```python
from build123d import *

# Parameters (mm, degrees)
SKETCH_1_W      = 26
SKETCH_1_H      = 12
SKETCH_1_W_2    = 20
SKETCH_1_H_2    = 8
EXTRUDE_1_DEPTH = 2.5
SKETCH_2_W      = 12
SKETCH_2_H      = 9
EXTRUDE_2_DEPTH = 2.5


with BuildPart() as part:
    # 草图1 → 凸台-拉伸1 (new, symmetric)
    with BuildSketch(Plane.XY):
        Rectangle(SKETCH_1_W, SKETCH_1_H)
        Rectangle(SKETCH_1_W_2, SKETCH_1_H_2, mode=Mode.SUBTRACT)
    extrude(amount=EXTRUDE_1_DEPTH, both=True)

    # 草图2 → 凸台-拉伸2 (add, symmetric)
    with BuildSketch(Plane.XY):
        with Locations((0, -10.5)):
            Rectangle(SKETCH_2_W, SKETCH_2_H)
    extrude(amount=EXTRUDE_2_DEPTH, both=True)


solid = part.part
```
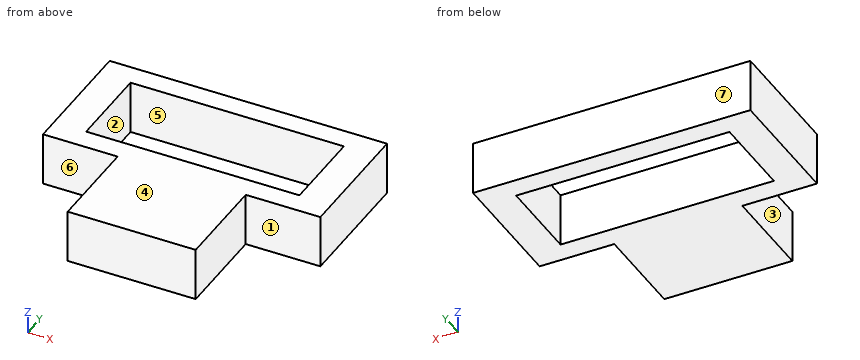
For this review, take the finished solid that the model builds, in its own axes (mm). Face numbers are marked on the shaded views. A direction names the side the tool comes from. Round coordinates to 2 decimals unless told otherwise and drop trailing zeros. Write each loop counter-clockwise with the first axis right and the second up, starting at its lowest first coordinate (ties: lowest second). Pieces come first, ordered by that corner, then holes.
1) Take a section at C-C on z = 0. Give the boundary of the cut face in (x, y), then the cut area to 3 significant figures.
Answer below:
outline: (-13, -6) - (-6, -6) - (-6, -15) - (6, -15) - (6, -6) - (13, -6) - (13, 6) - (-13, 6) - close; hole (-10, -4) - (10, -4) - (10, 4) - (-10, 4) - close
area: 260 mm2
2) Take a section at D-D on x = 10.75. Give the boundary of the cut face in (y, z).
Answer below:
outline: (-6, -2.5) - (6, -2.5) - (6, 2.5) - (-6, 2.5) - close
3) Take a section at B-B on y = 1.25. Give the boundary of the cut face in (x, z).
Answer below:
outline: (-13, -2.5) - (-10, -2.5) - (-10, 2.5) - (-13, 2.5) - close; (10, -2.5) - (13, -2.5) - (13, 2.5) - (10, 2.5) - close
4) Take a section at A-A on x = -3.75. Give the boundary of the cut face in (y, z).
Answer below:
outline: (-15, -2.5) - (-4, -2.5) - (-4, 2.5) - (-15, 2.5) - close; (4, -2.5) - (6, -2.5) - (6, 2.5) - (4, 2.5) - close
5) Machinability: for the marked faces 1, 2, 3 and 4, which of the approach directions +Z, -Z, +X, -X, +Y, -Y give a long, thin tool a straight path to every point of the face, cutting with its end or side? Answer none if there is none.
Answer below:
face 1: +Z, -Z, +X, -Y
face 2: +Z, -Z
face 3: +Z, -Z, -X, -Y
face 4: +Z, +X, -X, +Y, -Y
6) Mouldability with a two-part tool opening along Y and no side actions: class the marked faces 5, 6 and 7 as +Y half, -Y half, draft (parallel to the pull), parting line (faces both ways), or undercut.
Answer below:
face 5: undercut
face 6: -Y half
face 7: +Y half
7) Insertion check: pin 1 Ø4 at (x, y) = (1, -3) entering from -Z; pin 2 Ø1.5 at (x, z) = (-9, 1) entering from -Y. Each pin has a flat end and moves straight along its axis. Give the tip position at first contact, or say it passes through.
Answer below:
pin 1: stops at z = -2.5
pin 2: stops at y = -6
8) For line 1 along Y through (x, z) = (9, -0.5); line 2 along X through (y, z) = (2, 1.65); line 3 along X through (y, z) = (-8.25, 1.25), list the stretches that pass through material, from the lowest coordinate up.
Answer below:
line 1: y = -6 to -4, 4 to 6
line 2: x = -13 to -10, 10 to 13
line 3: x = -6 to 6
